Work out the finished part from the listing and answer in its coordinate system (mm). Face numbers are marked on the shaded views. A direction names the side the tool comes from. Coordinates: 2 decimals unless noted, no trailing zeros. Loops run counter-clockwise (first coordinate to the right, second up) from the corner with the lowest first, then second, coordinate; pieces in that order, holes last. Notation, with made-up numbers: (26.5, -2) -> (79.5, -2) arc R19 ccw to (79.5, 2) -> close; hole circle Ø7 at (24, 40.5). An arc over 180 degrees is marked (long way). Use a Markdown table: item, result.
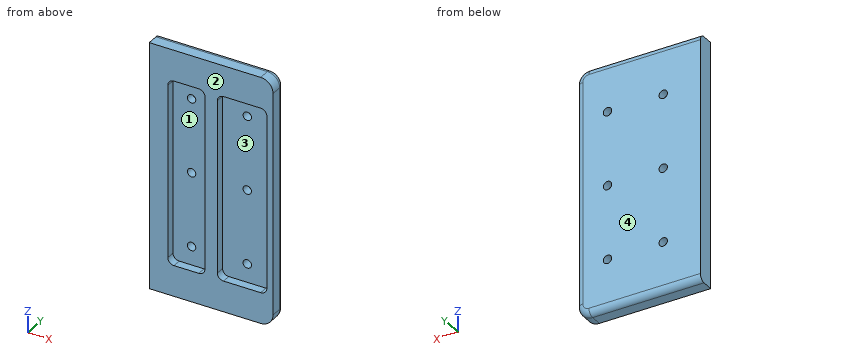
from build123d import *

# Parameters (mm, degrees)
SKETCH1_W                  = 100
SKETCH1_H                  = 200
BOSS_EXTRUDE1_DEPTH        = 14
FILLET1_R                  = 10
FILLET2_R                  = 5
SKETCH10_W                 = 40
SKETCH10_H                 = 150
BOSS_EXTRUDE3_DEPTH        = 3
SKETCH11_W                 = 10
SKETCH11_H                 = 150
CUT_EXTRUDE5_DEPTH         = 3
SKETCH12_W                 = 40
SKETCH12_H                 = 150
SKETCH12_W_2               = 30
CUT_EXTRUDE6_DEPTH         = 10
M8_TAPPED_HOLE2_AT_2_COUNT = 2
M8_TAPPED_HOLE2_AT_2_PITCH = 60
M8_TAPPED_HOLE2_AT_3_COUNT = 2
M8_TAPPED_HOLE2_AT_3_PITCH = 120
LPATTERN1_COUNT            = 2
LPATTERN1_PITCH            = 45
FILLET3_R                  = 5


with BuildPart() as part:
    # Sketch1 → Boss-Extrude1 (new body)
    with BuildSketch(Plane(origin=(0, 0, 0), x_dir=(1, 0, 0), z_dir=(0, 1, 0))):
        Rectangle(SKETCH1_W, SKETCH1_H)
    extrude(amount=BOSS_EXTRUDE1_DEPTH)

    # Fillet1
    fillet1_edges = [part.edges().sort_by_distance(p)[0] for p in [
        (50, 7, 100),
        (50, 7, -100),
    ]]
    fillet(fillet1_edges, radius=FILLET1_R)

    # Fillet2
    fillet2_edges = [part.edges().sort_by_distance(p)[0] for p in [
        (-5, 14, -100),
        (50, 14, 0),
        (-5, 14, 100),
        (47.071067812, 14, 97.071067812),
        (47.071067812, 14, -97.071067812),
    ]]
    fillet(fillet2_edges, radius=FILLET2_R)

    # Sketch10 → Boss-Extrude3 (add)
    with BuildSketch(Plane.XZ):
        with Locations((-25, 0)):
            Rectangle(SKETCH10_W, SKETCH10_H)
        with Locations((25, 0)):
            Rectangle(SKETCH10_W, SKETCH10_H)
    extrude(amount=BOSS_EXTRUDE3_DEPTH)

    # Sketch11 → Cut-Extrude5 (cut)
    with BuildSketch(Plane.XZ.offset(3)):
        with Locations((-40, 0)):
            Rectangle(SKETCH11_W, SKETCH11_H)
    extrude(amount=-CUT_EXTRUDE5_DEPTH, mode=Mode.SUBTRACT)

    # Sketch12 → Cut-Extrude6 (cut)
    with BuildSketch(Plane.XZ.offset(3)):
        with Locations((25, 0)):
            Rectangle(SKETCH12_W, SKETCH12_H)
        with Locations((-20, 0)):
            Rectangle(SKETCH12_W_2, SKETCH12_H)
    extrude(amount=-CUT_EXTRUDE6_DEPTH, mode=Mode.SUBTRACT)

    # Sketch14 → M8 Tapped Hole2 (revolve, cut)
    with BuildSketch(Plane(origin=(25, 7, -60), x_dir=(0, 0, -1), z_dir=(1, 0, 0))):
        Polygon((0, 0), (0, 21.792926105), (3.4, 19.75), (3.4, 0), align=None)
    m8_tapped_hole2 = revolve(axis=Axis((25, 0.65, -60), (0, 1, 0)), mode=Mode.SUBTRACT)

    # M8 Tapped Hole2 at 2: M8 Tapped Hole2 ×2
    with Locations(*[(0, 0, i * M8_TAPPED_HOLE2_AT_2_PITCH) for i in range(1, M8_TAPPED_HOLE2_AT_2_COUNT)]):
        add(m8_tapped_hole2, mode=Mode.SUBTRACT)

    # M8 Tapped Hole2 at 3: M8 Tapped Hole2 ×2
    with Locations(*[(0, 0, i * M8_TAPPED_HOLE2_AT_3_PITCH) for i in range(1, M8_TAPPED_HOLE2_AT_3_COUNT)]):
        add(m8_tapped_hole2, mode=Mode.SUBTRACT)

    # LPattern1: M8 Tapped Hole2 ×2
    with Locations(*[(-i * LPATTERN1_PITCH, 0, 0) for i in range(1, LPATTERN1_COUNT)]):
        add(m8_tapped_hole2, mode=Mode.SUBTRACT)

    # LPattern1 copy 1 sketch → LPattern1 copy 1 (revolve, cut)
    with BuildSketch(Plane(origin=(-20, 7, 0), x_dir=(0, 0, -1), z_dir=(1, 0, 0))):
        Polygon((0, 0), (0, 21.792926105), (3.4, 19.75), (3.4, 0), align=None)
    revolve(axis=Axis((-20, 0.65, 0), (0, 1, 0)), mode=Mode.SUBTRACT)

    # LPattern1 copy 2 sketch → LPattern1 copy 2 (revolve, cut)
    with BuildSketch(Plane(origin=(-20, 7, 60), x_dir=(0, 0, -1), z_dir=(1, 0, 0))):
        Polygon((0, 0), (0, 21.792926105), (3.4, 19.75), (3.4, 0), align=None)
    revolve(axis=Axis((-20, 0.65, 60), (0, 1, 0)), mode=Mode.SUBTRACT)

    # Fillet3
    fillet3_edges = [part.edges().sort_by_distance(p)[0] for p in [
        (45, 3.5, 75),
        (45, 3.5, -75),
        (5, 3.5, -75),
        (5, 3.5, 75),
        (-5, 3.5, 75),
        (-35, 3.5, -75),
        (-35, 3.5, 75),
        (-5, 3.5, -75),
    ]]
    fillet(fillet3_edges, radius=FILLET3_R)


solid = part.part
Q1. Given pin 1 Ø12 at (x, z) = (25, 16) entering from -Y; pin 2 Ø1.5 at (x, y) = (-7.5, 11.5) entering from +Z, each flat-ended and moving along its own axis, determine where each tip first touches the part or whether it passes through.
Solved:
| item | result |
|---|---|
| pin 1 | y = 7 |
| pin 2 | z = 99.68 |
Q2. Consider line 1 (X direction, y = 2.5, z = -28); line 2 (X direction, y = 9.25, z = 60); line 3 (Z direction, x = -20, y = 11.5). Determine where each line is inside the solid, lowest interval first. Write a range as [from, to].
Solved:
| item | result |
|---|---|
| line 1 | [-50, -35], [-5, 5], [45, 50] |
| line 2 | [-50, -23.4], [-16.6, 21.6], [28.4, 49.99] |
| line 3 | [-99.33, -63.4], [-56.6, -3.4], [3.4, 56.6], [63.4, 99.33] |
Q3. Section A-A on x = 25 is taken. Determine the outline of the cut face in (y, z).
Solved:
| item | result |
|---|---|
| outline | (0, -100) -> (9, -100) arc R5 ccw to (14, -95) -> (14, -63.4) -> (7, -63.4) -> (7, -75) -> (0, -75) -> close; (0, 75) -> (7, 75) -> (7, 63.4) -> (14, 63.4) -> (14, 95) arc R5 ccw to (9, 100) -> (0, 100) -> close; (7, -56.6) -> (14, -56.6) -> (14, -3.4) -> (7, -3.4) -> close; (7, 3.4) -> (14, 3.4) -> (14, 56.6) -> (7, 56.6) -> close |
Q4. Determine the mould class of the marked faces 1 and 2 for opening direction Z: pulls with the +Z half, pulls with the -Z half, needs draft (parallel to the pull), parting line crosses it, or undercut.
Solved:
| item | result |
|---|---|
| face 1 | undercut |
| face 2 | needs draft |
Q5. For the marked faces 3 and 4, determine the directions among +Z, -Z, +X, -X, +Y, -Y from which every point of the face is accessible in a straight line to the end or side of a thin tool.
Solved:
| item | result |
|---|---|
| face 3 | -Y |
| face 4 | +Z, -Z, +X, -X, +Y |
Q6. Section B-B on z = -60 is taken. Determine the outline of the cut face in (x, y), and give its area (3 significant figures).
Solved:
| item | result |
|---|---|
| outline | (-50, 0) -> (-35, 0) -> (-35, 7) -> (-23.4, 7) -> (-23.4, 14) -> (-50, 14) -> close; (-16.6, 7) -> (-5, 7) -> (-5, 0) -> (5, 0) -> (5, 7) -> (21.6, 7) -> (21.6, 14) -> (-16.6, 14) -> close; (28.4, 7) -> (45, 7) -> (45, 0) -> (50, 0) -> (50, 9) arc R5 ccw to (45, 14) -> (28.4, 14) -> close |
| area | 809 mm² |
Q7. Section C-C on y = 2 is taken. Determine the outline of the cut face in (x, z).
Solved:
| item | result |
|---|---|
| outline | (-50, -100) -> (40, -100) arc R10 ccw to (50, -90) -> (50, 90) arc R10 ccw to (40, 100) -> (-50, 100) -> close; hole (-35, -70) arc R5 ccw to (-30, -75) -> (-10, -75) arc R5 ccw to (-5, -70) -> (-5, 70) arc R5 ccw to (-10, 75) -> (-30, 75) arc R5 ccw to (-35, 70) -> close; hole (5, -70) arc R5 ccw to (10, -75) -> (40, -75) arc R5 ccw to (45, -70) -> (45, 70) arc R5 ccw to (40, 75) -> (10, 75) arc R5 ccw to (5, 70) -> close |
Q8. Section D-D on z = -7 is taken. Determine the outline of the cut face in (x, y), and give its area (3 significant figures).
Solved:
| item | result |
|---|---|
| outline | (-50, 0) -> (-35, 0) -> (-35, 7) -> (-5, 7) -> (-5, 0) -> (5, 0) -> (5, 7) -> (45, 7) -> (45, 0) -> (50, 0) -> (50, 9) arc R5 ccw to (45, 14) -> (-50, 14) -> close |
| area | 905 mm² |
